```python
from build123d import *

# Parameters (mm, degrees)
UNEQUAL_ANGLE_7_5_5_5_1_DEPTH = 2276
M6_TAPPED_HOLE2_D             = 5
M6_TAPPED_HOLE2_DEPTH         = 15
M6_TAPPED_HOLE2_TIP           = 1.502151548
M6_TAPPED_HOLE1_D             = 5
M6_TAPPED_HOLE1_DEPTH         = 15
M6_TAPPED_HOLE1_TIP           = 1.502151548
CUT_EXTRUDE1_DEPTH            = 10


with BuildPart() as part:
    # Sketch19 → Unequal angle 7.5-5-5(1) (new body)
    with BuildSketch(Plane.YZ.offset(-1138)):
        with BuildLine():
            Line((75, 0), (0, 0))
            Line((0, 0), (0, -50))
            Line((0, -50), (3.333333333, -50))
            ThreePointArc((3.333333333, -50), (4.511844635, -49.511844635), (5, -48.333333333))
            Line((5, -48.333333333), (5, -13))
            ThreePointArc((5, -13), (7.343145751, -7.343145751), (13, -5))
            Line((13, -5), (73.333333333, -5))
            ThreePointArc((73.333333333, -5), (74.511844635, -4.511844635), (75, -3.333333333))
            Line((75, -3.333333333), (75, 0))
        make_face()
    extrude(amount=UNEQUAL_ANGLE_7_5_5_5_1_DEPTH)

    # M6 Tapped Hole2
    with Locations(Plane(origin=(0, 5, 0), x_dir=(1, 0, 0), z_dir=(0, 1, 0))):
        with Locations((-591.5, 27), (-556.5, 27), (17.5, 27), (-17.5, 27), (591.5, 27), (556.5, 27)):
            Hole(M6_TAPPED_HOLE2_D / 2, depth=M6_TAPPED_HOLE2_DEPTH)
            with Locations((0, 0, -(M6_TAPPED_HOLE2_DEPTH + M6_TAPPED_HOLE2_TIP / 2))):  # 118° drill point
                Cone(0, M6_TAPPED_HOLE2_D / 2, M6_TAPPED_HOLE2_TIP, mode=Mode.SUBTRACT)

    # M6 Tapped Hole1
    with Locations(Plane(origin=(0, 0, -5), x_dir=(-1, 0, 0), z_dir=(0, 0, -1))):
        with Locations((17.5, 56.932613047), (-591.5, 56.932613047), (-556.5, 56.932613047), (-574, 30.932613047), (556.5, 56.932613047), (591.5, 56.932613047), (574, 30.932613047), (-17.5, 56.932613047), (0, 30.932613047)):
            Hole(M6_TAPPED_HOLE1_D / 2, depth=M6_TAPPED_HOLE1_DEPTH)
            with Locations((0, 0, -(M6_TAPPED_HOLE1_DEPTH + M6_TAPPED_HOLE1_TIP / 2))):  # 118° drill point
                Cone(0, M6_TAPPED_HOLE1_D / 2, M6_TAPPED_HOLE1_TIP, mode=Mode.SUBTRACT)

    # Sketch12 → Cut-Extrude1 (cut)
    with BuildSketch(Plane(origin=(0, 0, -5), x_dir=(-1, 0, 0), z_dir=(0, 0, -1))):
        with BuildLine():
            Line((1128, 53), (1120, 53))
            ThreePointArc((1120, 53), (1115, 58), (1120, 63))
            Line((1120, 63), (1128, 63))
            ThreePointArc((1128, 63), (1133, 58), (1128, 53))
        make_face()
        with BuildLine():
            Line((1120, 33), (1128, 33))
            ThreePointArc((1128, 33), (1133, 28), (1128, 23))
            Line((1128, 23), (1120, 23))
            ThreePointArc((1120, 23), (1115, 28), (1120, 33))
        make_face()
        with BuildLine():
            Line((-1128, 63), (-1120, 63))
            ThreePointArc((-1120, 63), (-1115, 58), (-1120, 53))
            Line((-1120, 53), (-1128, 53))
            ThreePointArc((-1128, 53), (-1133, 58), (-1128, 63))
        make_face()
        with BuildLine():
            Line((-1128, 33), (-1120, 33))
            ThreePointArc((-1120, 33), (-1115, 28), (-1120, 23))
            Line((-1120, 23), (-1128, 23))
            ThreePointArc((-1128, 23), (-1133, 28), (-1128, 33))
        make_face()
    extrude(amount=-CUT_EXTRUDE1_DEPTH, mode=Mode.SUBTRACT)


solid = part.part
```
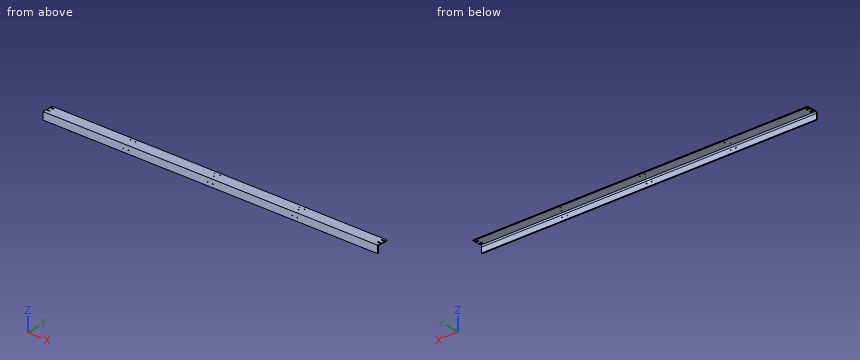
Build history of the part. All positions in model axes, mm. Round coordinates to 2 decimals unless told otherwise and drop trailing zeros. Loops run counter-clockwise (first coordinate to the right, second up) from the corner with the lowest first, then second, coordinate; pieces in that order, holes last.
Item 1: Pin check, flat tips, straight feed: P1, Ø8, axis at x = -17.5, z = -27, coming from the +Y side; P2, Ø4, axis at x = 556.5, y = 56.93, coming from the +Z side; P3, Ø4, axis at x = -873.5, y = 67, coming from the -Z side. Stop position of each tip, or through.
Item 2: Drill centre lines: line 1 along Y through (x, z) = (-17, -2); line 2 along Z through (x, y) = (591, 2); line 3 along Z through (x, y) = (-17.5, 3.55). Where is each one in solid material? Low to high.
Item 3: Saw through at A-A (x = 71.5). List the corners of the cut face in (y, z).
Worked answers:
1. P1: stops at y = 5
1. P2: passes through
1. P3: stops at z = -5
2. line 1: y = 0 to 54.48, 59.38 to 75
2. line 2: z = -50 to -29.45, -24.55 to 0
2. line 3: z = -49.99 to -29.5, -24.5 to 0
3. outline: (0, -50) - (3.33, -50) arc R1.67 ccw to (5, -48.33) - (5, -13) arc R8 cw to (13, -5) - (73.33, -5) arc R1.67 ccw to (75, -3.33) - (75, 0) - (0, 0) - close
